Design review of the part built by this model. Coordinates are the model's own, in mm. A direction names the side the tool comes from. Coordinates: 2 decimals unless noted, no trailing zeros. Write each loop counter-clockwise with the first axis right and the second up, starting at its lowest first coordinate (ties: lowest second). Pieces come first, ordered by that corner, then holes. Notation, with made-up numbers: (5, 19.5) - (39, 19.5) arc R19 cw to (39, 38.5) - close; hole circle Ø10 at (47.25, 84). An arc over 180 degrees is marked (long way). Answer as a JSON object with one key per item and string values.
```python
from build123d import *

# Parameters (mm, degrees)
SKETCH_1_R      = 3.25
SKETCH_1_R_2    = 1.25
EXTRUDE_1_DEPTH = 4
FILLET_1_R      = 1
FILLET_2_R      = 2
FILLET_3_R      = 3


with BuildPart() as part:
    # 草图1 → 凸台-拉伸1 (new body)
    # profile 1 of 12: a face of its own
    with BuildSketch(Plane(origin=(0, 0, 0), x_dir=(1, 0, 0), z_dir=(0, 1, 0))):
        with Locations((-10, 40)):
            Circle(SKETCH_1_R)
        with Locations(Location((-10, 40, 0), (0, 0, 270))):
            Circle(SKETCH_1_R_2, mode=Mode.SUBTRACT)
    # profile 2 of 12: a face of its own
    with BuildSketch(Plane(origin=(0, 0, 0), x_dir=(1, 0, 0), z_dir=(0, 1, 0))):
        with BuildLine():
            Line((-8.603139344, 37.065501694), (-3.516561637, 34.522212841))
            Line((-3.516561637, 34.522212841), (-3.12495283, 35.892843666))
            ThreePointArc((-3.12495283, 35.892843666), (-2.480682914, 37.099693378), (-1.396860656, 37.934498306))
            Line((-1.396860656, 37.934498306), (-6.814284962, 40.643210458))
            ThreePointArc((-6.814284962, 40.643210458), (-6.766111174, 40.32320746), (-6.75, 40))
            ThreePointArc((-6.75, 40), (-7.252064672, 38.26467541), (-8.603139344, 37.065501694))
        make_face()
    # profile 3 of 12: a face of its own
    with BuildSketch(Plane(origin=(0, 0, 0), x_dir=(1, 0, 0), z_dir=(0, 1, 0))):
        with BuildLine():
            ThreePointArc((-13.12495283, 0.892843666), (-11.578339526, 2.841011147), (-9.107156334, 3.12495283))
            Line((-9.107156334, 3.12495283), (-0.892843666, 31.87504717))
            ThreePointArc((-0.892843666, 31.87504717), (-2.38713669, 32.79453442), (-3.185715038, 34.356789542))
            Line((-3.185715038, 34.356789542), (-3.516561637, 34.522212841))
            Line((-3.516561637, 34.522212841), (-13.12495283, 0.892843666))
        make_face()
    # profile 4 of 12: a face of its own
    with BuildSketch(Plane(origin=(0, 0, 0), x_dir=(1, 0, 0), z_dir=(0, 1, 0))):
        with BuildLine():
            ThreePointArc((3.185715038, 34.356789542), (2.38713669, 32.79453442), (0.892843666, 31.87504717))
            Line((0.892843666, 31.87504717), (9.107156334, 3.12495283))
            ThreePointArc((9.107156334, 3.12495283), (11.578339526, 2.841011147), (13.12495283, 0.892843666))
            Line((13.12495283, 0.892843666), (3.516561637, 34.522212841))
            Line((3.516561637, 34.522212841), (3.185715038, 34.356789542))
        make_face()
    # profile 5 of 12: a face of its own
    with BuildSketch(Plane(origin=(0, 0, 0), x_dir=(1, 0, 0), z_dir=(0, 1, 0))):
        with Locations((-10, 0)):
            Circle(SKETCH_1_R)
        with Locations(Location((-10, 0, 0), (0, 0, 270))):
            Circle(SKETCH_1_R_2, mode=Mode.SUBTRACT)
    # profile 6 of 12: a face of its own
    with BuildSketch(Plane(origin=(0, 0, 0), x_dir=(1, 0, 0), z_dir=(0, 1, 0))):
        with BuildLine():
            Line((6.75, 0), (-6.75, 0))
            ThreePointArc((-6.75, 0), (-7.701902961, -2.298097039), (-10, -3.25))
            Line((-10, -3.25), (10, -3.25))
            ThreePointArc((10, -3.25), (7.701902961, -2.298097039), (6.75, 0))
        make_face()
    # profile 7 of 12: a face of its own
    with BuildSketch(Plane(origin=(0, 0, 0), x_dir=(1, 0, 0), z_dir=(0, 1, 0))):
        with Locations((10, 0)):
            Circle(SKETCH_1_R)
        with Locations(Location((10, 0, 0), (0, 0, 270))):
            Circle(SKETCH_1_R_2, mode=Mode.SUBTRACT)
    # profile 8 of 12: a face of its own
    with BuildSketch(Plane(origin=(0, 0, 0), x_dir=(1, 0, 0), z_dir=(0, 1, 0))):
        with Locations((0, 35)):
            Circle(SKETCH_1_R)
        with Locations(Location((0, 35, 0), (0, 0, 270))):
            Circle(SKETCH_1_R_2, mode=Mode.SUBTRACT)
    # profile 9 of 12: a face of its own
    with BuildSketch(Plane(origin=(0, 0, 0), x_dir=(1, 0, 0), z_dir=(0, 1, 0))):
        with BuildLine():
            Line((-3.516561637, 34.522212841), (-3.185715038, 34.356789542))
            ThreePointArc((-3.185715038, 34.356789542), (-3.247460208, 35.128460874), (-3.12495283, 35.892843666))
            Line((-3.12495283, 35.892843666), (-3.516561637, 34.522212841))
        make_face()
    # profile 10 of 12: a face of its own
    with BuildSketch(Plane(origin=(0, 0, 0), x_dir=(1, 0, 0), z_dir=(0, 1, 0))):
        with BuildLine():
            ThreePointArc((3.25, 35), (3.233888826, 34.67679254), (3.185715038, 34.356789542))
            Line((3.185715038, 34.356789542), (3.516561637, 34.522212841))
            Line((3.516561637, 34.522212841), (3.12495283, 35.892843666))
            ThreePointArc((3.12495283, 35.892843666), (3.21858639, 35.450778939), (3.25, 35))
        make_face()
    # profile 11 of 12: a face of its own
    with BuildSketch(Plane(origin=(0, 0, 0), x_dir=(1, 0, 0), z_dir=(0, 1, 0))):
        with BuildLine():
            Line((3.12495283, 35.892843666), (3.516561637, 34.522212841))
            Line((3.516561637, 34.522212841), (8.603139344, 37.065501694))
            ThreePointArc((8.603139344, 37.065501694), (7.093111629, 38.546555815), (6.814284962, 40.643210458))
            Line((6.814284962, 40.643210458), (1.396860656, 37.934498306))
            ThreePointArc((1.396860656, 37.934498306), (2.480682914, 37.099693378), (3.12495283, 35.892843666))
        make_face()
    # profile 12 of 12: a face of its own
    with BuildSketch(Plane(origin=(0, 0, 0), x_dir=(1, 0, 0), z_dir=(0, 1, 0))):
        with Locations((10, 40)):
            Circle(SKETCH_1_R)
        with Locations(Location((10, 40, 0), (0, 0, 270))):
            Circle(SKETCH_1_R_2, mode=Mode.SUBTRACT)
    extrude(amount=EXTRUDE_1_DEPTH)

    # 圆角1
    fillet_1_edges = [part.edges().sort_by_distance(p)[0] for p in [
        (9.107156334, 2, -3.12495283),
        (0.892843666, 2, -31.87504717),
        (-0.892843666, 2, -31.87504717),
        (-9.107156334, 2, -3.12495283),
        (-6.75, 2, 0),
        (6.75, 2, 0),
    ]]
    fillet(fillet_1_edges, radius=FILLET_1_R)

    # 圆角2
    fillet_2_edges = [part.edges().sort_by_distance(p)[0] for p in [
        (-3.516561637, 2, -34.522212841),
        (-1.396860656, 2, -37.934498306),
        (1.396860656, 2, -37.934498306),
        (3.516561637, 2, -34.522212841),
    ]]
    fillet(fillet_2_edges, radius=FILLET_2_R)

    # 圆角3
    fillet_3_edges = [part.edges().sort_by_distance(p)[0] for p in [
        (-8.603139344, 2, -37.065501694),
        (-6.814284962, 2, -40.643210458),
        (6.814284962, 2, -40.643210458),
        (8.603139344, 2, -37.065501694),
    ]]
    fillet(fillet_3_edges, radius=FILLET_3_R)


solid = part.part
```
(1) The part is to be moulded in two halves that separate along Z. For faces 1 (the face through (7.417, 1.972, -1.972)), 2 (the face through (6.52, 2.03, -40.66)), say which applies: pulls with the +Z half, pulls with the -Z half, needs draft (parallel to the pull), parting line crosses it, or undercut.
Solved:
{"face 1": "undercut", "face 2": "pulls with the -Z half"}
(2) To check wall thickness, follow line 1 (X direction, y = 0.8, z = -40); line 2 (X direction, y = 2.3, z = -31.5); line 3 (X direction, y = 1.2, z = -27.5). State the ranges of each line that lie inside material, in increasing order. Write a range as from..to.
Solved:
{"line 1": "x = -13.25..-11.25, -8.75..-5.53, 5.53..8.75, 11.25..13.25", "line 2": "x = -4.38..-0.84, 0.84..4.38", "line 3": "x = -5.52..-2.14, 2.14..5.52"}
(3) Take a section at B-B, the plane x = 10.5. Write out the cut boundary in (y, z), and give its area (3 significant figures).
Solved:
{"outline": "(0, -43.21) - (4, -43.21) - (4, -41.15) - (0, -41.15) - close; (0, -38.85) - (4, -38.85) - (4, -36.79) - (0, -36.79) - close; (0, -10.08) - (4, -10.08) - (4, -1.15) - (0, -1.15) - close; (0, 1.15) - (4, 1.15) - (4, 3.21) - (0, 3.21) - close", "area": "60.5 mm^2"}
(4) Tool access review of faces 3 (the face through (-3.924, 1.972, -39.198)), 4 (the face through (4.057, 2.028, -34.263)), 5 (the face through (-8.471, 2.028, -36.823)): name each direction out of +Z, -Z, +X, -X, +Y, -Y from which nothing blocks a thin tool from reaching the whole face with its end or side.
Solved:
{"face 3": "-Z, +Y, -Y", "face 4": "+X, +Y, -Y", "face 5": "+Y, -Y"}
(5) For pin 1 (1.5 mm diameter, centred on x = 4.5, y = 3, fed in from -Z), flat-tipped, find the tip position at first contact; note if it passes through.
Solved:
{"pin 1": "stops at z = -39.86"}
(6) Take a section at A-A, the plane z = -15.5. Write out the cut boundary in (x, y), and give its area (3 significant figures).
Solved:
{"outline": "(-8.95, 0) - (-5.57, 0) - (-5.57, 4) - (-8.95, 4) - close; (5.57, 0) - (8.95, 0) - (8.95, 4) - (5.57, 4) - close", "area": "27.0 mm^2"}
(7) Take a section at D-D, the plane y = 1.7. Give the number of separate pieces and of enclosed holes in the cut face, and give its area (3 significant figures).
Solved:
{"separate pieces": "1", "enclosed holes": "6", "area": "437 mm^2"}
(8) Take a section at C-C, the plane z = -2. Write out the cut boundary in (x, y).
Solved:
{"outline": "(-12.81, 0) - (-7.44, 0) - (-7.44, 4) - (-12.81, 4) - close; (7.44, 0) - (12.81, 0) - (12.81, 4) - (7.44, 4) - close"}
